Input: part model. Units: mm. Frame: model coordinates. Face numbers are marked on the shaded views. Give positions to 0.01 mm unless a question says otherwise; leave off trailing zeros. Loops run counter-clockwise (first coordinate to the right, second up) from the corner with the lowest first, then second, coordinate; pieces in that order, holes last. Notation, with made-up numbers: (9, 59) -> (29, 59) arc R16 cw to (29, 78) -> close; hole circle Ø5 at (86.25, -37.75). An arc over 180 degrees is marked (long way). Answer in a Markdown table with one row per item. Add a question column.
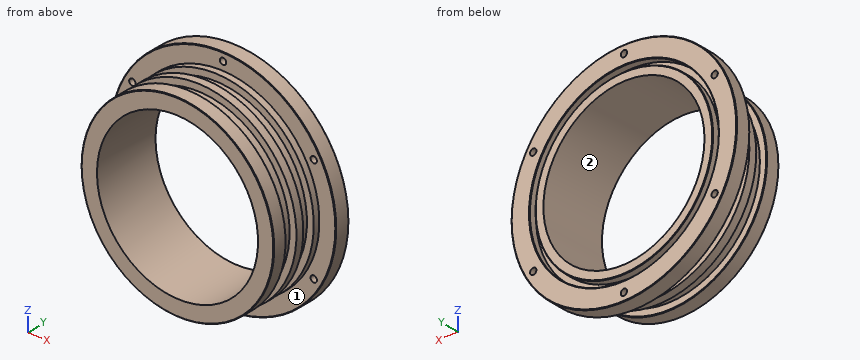
```python
from build123d import *

# Parameters (mm, degrees)
CHAMFER_1_SIZE         = 0.2
HOLE_WIZARD_M3_1_D     = 2.5
HOLE_WIZARD_M3_1_DEPTH = 7.5
HOLE_WIZARD_M3_1_TIP   = 0.751075774
SKETCH_4_R             = 37.25
SKETCH_4_R_2           = 35
CUT_EXTRUDE_1_DEPTH    = 3
CHAMFER_2_SIZE         = 0.2


with BuildPart() as part:
    # 草图1 → 旋转1 (revolve)
    with BuildSketch(Plane.XY):
        Polygon((-31.75, 27), (-31.75, 0), (-37.973, 0), (-37.973, 5.587), (-35.2806, 5.587), (-35.2806, 10.413), (-37.973, 10.413), (-37.973, 13.587), (-35.2806, 13.587), (-35.2806, 18.413), (-37.973, 18.413), (-37.973, 21), (-44.45, 21), (-44.45, 27), align=None)
    revolve(axis=Axis((0, 27, 0), (0, -1, 0)))

    # 倒角1
    chamfer_1_edges = [part.edges().sort_by_distance(p)[0] for p in [
        (37.973, 5.587, 0),
        (37.973, 0, 0),
        (44.45, 27, 0),
        (44.45, 21, 0),
    ]]
    chamfer(chamfer_1_edges, length=CHAMFER_1_SIZE)

    # M3 螺纹孔1
    with Locations(Plane(origin=(0, 27, 0), x_dir=(1, 0, 0), z_dir=(0, 1, 0))):
        with Locations((-35.745198541, -20.6375), (-35.745198541, 20.6375), (0, 41.275), (35.745198541, 20.6375), (35.745198541, -20.6375), (0, -41.275)):
            Hole(HOLE_WIZARD_M3_1_D / 2, depth=HOLE_WIZARD_M3_1_DEPTH)
            with Locations((0, 0, -(HOLE_WIZARD_M3_1_DEPTH + HOLE_WIZARD_M3_1_TIP / 2))):  # 118° drill point
                Cone(0, HOLE_WIZARD_M3_1_D / 2, HOLE_WIZARD_M3_1_TIP, mode=Mode.SUBTRACT)

    # 草图4 → 切除-拉伸1 (cut)
    with BuildSketch(Plane(origin=(0, 27, 0), x_dir=(1, 0, 0), z_dir=(0, 1, 0))):
        with Locations(Location((0, 0, 0), (0, 0, 180))):
            Circle(SKETCH_4_R)
        with Locations(Location((0, 0, 0), (0, 0, 180))):
            Circle(SKETCH_4_R_2, mode=Mode.SUBTRACT)
    extrude(amount=-CUT_EXTRUDE_1_DEPTH, mode=Mode.SUBTRACT)

    # 倒角2
    chamfer_2_edges = [part.edges().sort_by_distance(p)[0] for p in [
        (37.25, 27, 0),
        (35, 27, 0),
    ]]
    chamfer(chamfer_2_edges, length=CHAMFER_2_SIZE)


solid = part.part
```
1) Pull-direction query (X, two-part tool) for the marked faces 1 and 2; classes: +X half, -X half, draft (parallel to the pull), parting line (faces both ways), or undercut.
2) Pin query (flat end, axial travel): pin 1 (12 mm diameter, centred on y = 7.5, z = -23, fed in from -X); pin 2 (12 mm diameter, centred on x = 32.5, y = 8, fed in from -Z); pin 3 (4 mm diameter, centred on x = -20, z = 35, fed in from -Y). Return the tip coordinate at first contact, or that it passes through.
3) Section A-A on y = 15.5. Output: boundary loops of the cut face in (x, z), and give its area (3 significant figures).
4) Material intervals for line 1 along Z through (x, y) = (0, 25) (3 decimals); line 2 along Z through (x, y) = (-20, 25.5); line 3 along X through (y, z) = (25.5, -18), sorted ascending.
5) Section B-B on x = 0. State how many separate pieces and enclosed holes the cut face has, and give its area (3 significant figures).
Working result:
| question | item | result |
|---|---|---|
| 1 | face 1 | draft |
| 1 | face 2 | undercut |
| 2 | pin 1 | stops at x = -33.76 |
| 2 | pin 2 | stops at z = -26.69 |
| 2 | pin 3 | stops at y = 21 |
| 3 | outline | circle Ø70.56 at (0, 0); hole circle Ø63.5 at (0, 0) |
| 3 | area | 743 mm2 |
| 4 | line 1 | z = -44.45 to -42.525, -40.025 to -37.25, -35 to -31.75, 31.75 to 35, 37.25 to 40.025, 42.525 to 44.45 |
| 4 | line 2 | z = -39.7 to -31.43, -28.72 to -24.66, 24.66 to 28.72, 31.43 to 39.7 |
| 4 | line 3 | x = -40.64 to -32.61, -30.02 to -26.15, 26.15 to 30.02, 32.61 to 40.64 |
| 5 | separate pieces | 4 |
| 5 | enclosed holes | 0 |
| 5 | area | 318 mm2 |
